Can you work these out from the drawing? Everything is in mm from the part's minimum corner. Coordinates: 2 decimals unless noted, no trailing zeros. Loops run counter-clockwise (first coordinate to the right, second up) from the corner with the lowest first, then second, coordinate; pieces in that order, holes last. Notation, with made-up numbers: M 30,84.5 L 77,84.5 A7 cw 77,95.5 Z; hole C 84.25,44 d9. An arc over 180 degrees is marked long. Use CSV: the item, a comma, the result in double quotes. Start each with the question number.
Q1. If we mould it in two halves opening along X, with no side actions, what happens to the marked faces 1, 2, 3 and 4? For each: +X half, -X half, draft (parallel to the pull), parting line (faces both ways), or undercut.
Q2. Please list where these lines run through material, in increasing order: probe 1 along Y at (x, z) = (11, 4.25); probe 2 along X at (y, z) = (12.5, 11.75); probe 3 along Y at (x, z) = (14.5, 11.5). Write a range as [from, to].
Q3. If we section it at C-C (z = 9.5): Please give me the cut outline in (x, y).
Q4. If we section it at A-A (y = 11): Please give me the cut outline in (x, z).
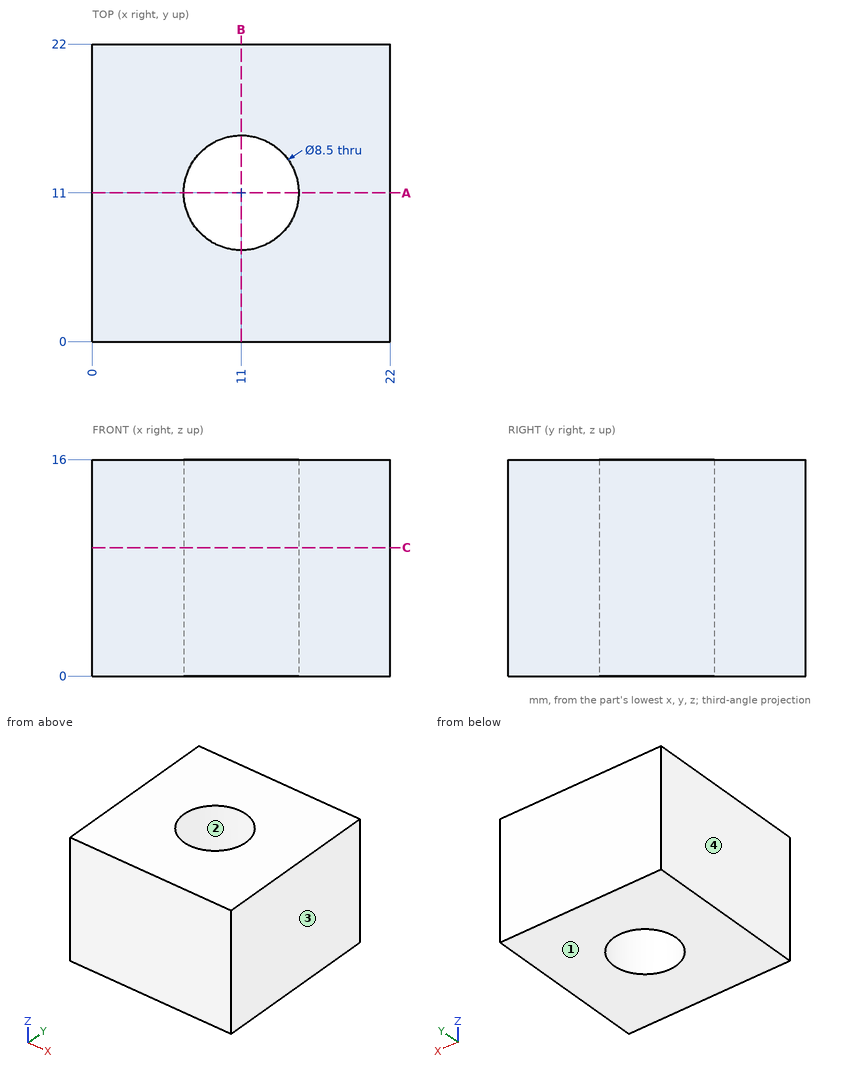
Results below:
1,face 1,"draft"
1,face 2,"undercut"
1,face 3,"+X half"
1,face 4,"-X half"
2,probe 1,"[0, 6.75], [15.25, 22]"
2,probe 2,"[0, 7.02], [14.98, 22]"
2,probe 3,"[0, 8.59], [13.41, 22]"
3,outline,"M 0,0 L 22,0 L 22,22 L 0,22 Z; hole C 11,11 d8.5"
4,outline,"M 0,0 L 6.75,0 L 6.75,16 L 0,16 Z; M 15.25,0 L 22,0 L 22,16 L 15.25,16 Z"
